```python
from build123d import *

# Parameters (mm, degrees)
SKETCH1_W              = 357
SKETCH1_H              = 60
BOSS_EXTRUDE1_DEPTH    = 76
SKETCH2_W              = 66.2
SKETCH2_H              = 36
CUT_EXTRUDE1_DEPTH     = 197.311614532
SKETCH3_R              = 23
CUT_EXTRUDE2_DEPTH     = 197.311614532
FILLET1_R              = 4
LPATTERN1_COUNT        = 4
LPATTERN1_PITCH        = 80
FILLET1_OF_LPATTERN1_R = 4


with BuildPart() as part:
    # Sketch1 → Boss-Extrude1 (new body)
    with BuildSketch(Plane.XY):
        Rectangle(SKETCH1_W, SKETCH1_H)
    extrude(amount=BOSS_EXTRUDE1_DEPTH)

    # Sketch2 → Cut-Extrude1 (cut, through all)
    with BuildSketch(Plane.XY.offset(76)):
        with Locations((-115.4, 32)):
            Rectangle(SKETCH2_W, SKETCH2_H)
    cut_extrude1 = extrude(amount=-CUT_EXTRUDE1_DEPTH, mode=Mode.SUBTRACT)

    # Sketch3 → Cut-Extrude2 (cut, through all)
    with BuildSketch(Plane.XY.offset(76)):
        with Locations((-115.4, 14)):
            Circle(SKETCH3_R)
    cut_extrude2 = extrude(amount=-CUT_EXTRUDE2_DEPTH, mode=Mode.SUBTRACT)

    # Fillet1
    fillet1_edges = [part.edges().sort_by_distance(p)[0] for p in [
        (-138.4, 14, 38),
        (-92.4, 14, 38),
    ]]
    fillet(fillet1_edges, radius=FILLET1_R)

    # LPattern1: Cut-Extrude1, Cut-Extrude2 ×4
    with Locations(*[(i * LPATTERN1_PITCH, 0, 0) for i in range(1, LPATTERN1_COUNT)]):
        add(cut_extrude1, mode=Mode.SUBTRACT)
        add(cut_extrude2, mode=Mode.SUBTRACT)

    # Fillet1 of LPattern1
    fillet1_of_lpattern1_edges = [part.edges().sort_by_distance(p)[0] for p in [
        (-58.4, 14, 38),
        (-12.4, 14, 38),
        (21.6, 14, 38),
        (67.6, 14, 38),
        (101.6, 14, 38),
        (147.6, 14, 38),
    ]]
    fillet(fillet1_of_lpattern1_edges, radius=FILLET1_OF_LPATTERN1_R)


solid = part.part
```
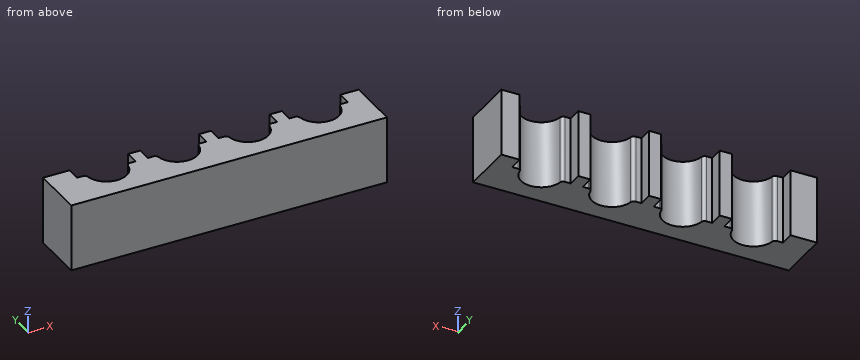
Source: CAD feature listing. Evaluate the final solid. Frame: model axes, mm. Give positions to 0.01 mm unless a question says otherwise; leave off trailing zeros. Write each loop counter-clockwise with the first axis right and the second up, starting at its lowest first coordinate (ties: lowest second). Pieces come first, ordered by that corner, then holes. Notation, with made-up numbers: (41, -16.75) - (99, -16.75) arc R21 cw to (99, 0.25) - close; hole circle Ø9 at (65, 22.25). An arc over 180 degrees is marked (long way). One line per item, written item: value. Start each with the question number.
Q1. Section query D-D, the plane x = 123. Return the cut outline in (y, z), then the cut area to 3 significant figures.
Q2. Material intervals for probe 1 along X at (y, z) = (10.5, 50); probe 2 along X at (y, z) = (18, 35); probe 3 along Y at (x, z) = (45, 31), sorted ascending. Write a range as from..to.
Q3. Section query B-B, the plane y = 5.5. Return the cut outline in (x, z), then the cut area to 3 significant figures.
Q4. Section query A-A, the plane y = 25.5. Return the cut outline in (x, z), then the cut area to 3 significant figures.
Q5. Section query C-C, the plane x = -129. Return the cut outline in (y, z).
Q6. First-contact query: pin 1 Ø8 at (x, z) = (-54.5, 45) entering from +Y; pin 2 Ø3 at (x, z) = (-4.5, 23.5) entering from +Y. Flat tips, straight axial feed; report the tip coordinate or a pass-through.
Answer:
1. outline: (-30, 0) - (-8.94, 0) - (-8.94, 76) - (-30, 76) - close
1. area: 1,600 mm2
2. probe 1: x = -178.5..-138.13, -92.67..-58.13, -12.67..21.87, 67.33..101.87, 147.33..178.5
2. probe 2: x = -178.5..-148.5, -82.3..-68.5, -2.3..11.5, 77.7..91.5, 157.7..178.5
2. probe 3: y = -30..-9
3. outline: (-178.5, 0) - (-136.77, 0) - (-136.77, 76) - (-178.5, 76) - close; (-94.03, 0) - (-56.77, 0) - (-56.77, 76) - (-94.03, 76) - close; (-14.03, 0) - (23.23, 0) - (23.23, 76) - (-14.03, 76) - close; (65.97, 0) - (103.23, 0) - (103.23, 76) - (65.97, 76) - close; (145.97, 0) - (178.5, 0) - (178.5, 76) - (145.97, 76) - close
3. area: 14,100 mm2
4. outline: (-178.5, 0) - (-148.5, 0) - (-148.5, 76) - (-178.5, 76) - close; (-82.3, 0) - (-68.5, 0) - (-68.5, 76) - (-82.3, 76) - close; (-2.3, 0) - (11.5, 0) - (11.5, 76) - (-2.3, 76) - close; (77.7, 0) - (91.5, 0) - (91.5, 76) - (77.7, 76) - close; (157.7, 0) - (178.5, 0) - (178.5, 76) - (157.7, 76) - close
4. area: 7,010 mm2
5. outline: (-30, 0) - (-4.55, 0) - (-4.55, 76) - (-30, 76) - close
6. pin 1: stops at y = 11.74
6. pin 2: stops at y = 14
